CAD build for the part. Positions are in the model's coordinates, mm. Coordinates: 2 decimals unless noted, no trailing zeros. Order: outer loops, then holes, each group sorted by start corner. A loop starts at its lowest first (then second) coordinate and runs counter-clockwise, first axis right, second up. Notation, with made-up numbers: (29.5, -15) - (38.5, -15) arc R26 ccw to (38.5, -1) - close; hole circle Ø1 at (-38.75, -6). An arc over 180 degrees is marked (long way). Write each question's results on one line, items separated by ' | '. Start each with the question number.
Q1. Band-saw the part on C-C, the plane z = 1.2. Write the cut outline in (x, y), then the cut area to 3 significant figures.
Q2. Band-saw the part on A-A, the plane x = -88. Write the cut outline in (y, z).
Q3. Band-saw the part on B-B, the plane y = 0. Write the cut outline in (x, z).
Q4. Wall check: probe 1 along Y at (x, z) = (-40, 1.5); probe 2 along Y at (x, z) = (-70.5, 1.1); probe 3 along X at (y, z) = (-0.5, 0.35). Give the ranges that are in metal, low to high.
Q5. Band-saw the part on D-D, the plane x = -40. Write the cut outline in (y, z), then the cut area to 3 significant figures.
Q6. Pin check, flat tips, straight feed: P1, Ø10.5, axis at x = 40, y = 0, coming from the -Z side; P2, Ø7, axis at x = -40, y = 0, coming from the +Z side. Stop position of each tip, or through.
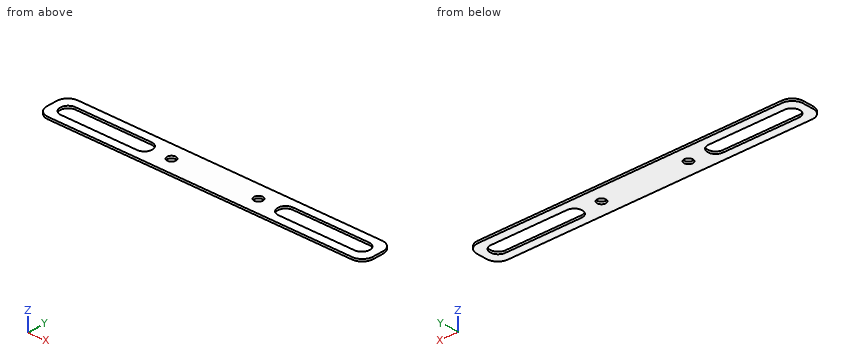
```python
from build123d import *

# Parameters (mm, degrees)
SKETCH1_W           = 300
SKETCH1_H           = 30
BOSS_EXTRUDE1_DEPTH = 2
CUT_EXTRUDE1_DEPTH  = 151.761400896
FILLET1_R           = 10
FILLET2_R           = 10
SKETCH4_R           = 4
CUT_EXTRUDE2_DEPTH  = 151.761400896


with BuildPart() as part:
    # Sketch1 → Boss-Extrude1 (new body)
    with BuildSketch(Plane.XY):
        Rectangle(SKETCH1_W, SKETCH1_H)
    extrude(amount=BOSS_EXTRUDE1_DEPTH)

    # Sketch2 → Cut-Extrude1 (cut, through all)
    with BuildSketch(Plane.XY.offset(2)):
        with BuildLine():
            Line((-135, 7.2), (-65, 7.2))
            ThreePointArc((-65, 7.2), (-57.8, 0), (-65, -7.2))
            Line((-65, -7.2), (-135, -7.2))
            ThreePointArc((-135, -7.2), (-142.2, 0), (-135, 7.2))
        make_face()
    cut_extrude1 = extrude(amount=-CUT_EXTRUDE1_DEPTH, mode=Mode.SUBTRACT)

    # Fillet1
    fillet1_edges = [part.edges().sort_by_distance(p)[0] for p in [
        (-150, 15, 1),
        (-150, -15, 1),
    ]]
    fillet(fillet1_edges, radius=FILLET1_R)

    # Mirror1: Cut-Extrude1 across plane
    add(cut_extrude1.mirror(Plane(origin=(0, 0, 0), x_dir=(0, 0, 1), z_dir=(1, 0, 0))), mode=Mode.SUBTRACT)

    # Fillet2
    fillet2_edges = [part.edges().sort_by_distance(p)[0] for p in [
        (150, 15, 1),
        (150, -15, 1),
    ]]
    fillet(fillet2_edges, radius=FILLET2_R)

    # Sketch4 → Cut-Extrude2 (cut, through all)
    with BuildSketch(Plane(origin=(0, 0, 0), x_dir=(-1, 0, 0), z_dir=(0, 0, -1))):
        with Locations((40, 0)):
            Circle(SKETCH4_R)
        with Locations((-40, 0)):
            Circle(SKETCH4_R)
    extrude(amount=-CUT_EXTRUDE2_DEPTH, mode=Mode.SUBTRACT)


solid = part.part
```
Results below:
1) outline: (-150, -5) arc R10 ccw to (-140, -15) - (140, -15) arc R10 ccw to (150, -5) - (150, 5) arc R10 ccw to (140, 15) - (-140, 15) arc R10 ccw to (-150, 5) - close; hole (-135, -7.2) - (-65, -7.2) arc R7.2 ccw to (-65, 7.2) - (-135, 7.2) arc R7.2 ccw to start; hole circle Ø8 at (-40, 0); hole circle Ø8 at (40, 0); hole (65, -7.2) - (135, -7.2) arc R7.2 ccw to (135, 7.2) - (65, 7.2) arc R7.2 ccw to start | area: 6,470 mm²
2) outline: (-15, 0) - (-7.2, 0) - (-7.2, 2) - (-15, 2) - close; (7.2, 0) - (15, 0) - (15, 2) - (7.2, 2) - close
3) outline: (-150, 0) - (-142.2, 0) - (-142.2, 2) - (-150, 2) - close; (-57.8, 0) - (-44, 0) - (-44, 2) - (-57.8, 2) - close; (-36, 0) - (36, 0) - (36, 2) - (-36, 2) - close; (44, 0) - (57.8, 0) - (57.8, 2) - (44, 2) - close; (142.2, 0) - (150, 0) - (150, 2) - (142.2, 2) - close
4) probe 1: y = -15 to -4, 4 to 15 | probe 2: y = -15 to -7.2, 7.2 to 15 | probe 3: x = -150 to -142.18, -57.82 to -43.97, -36.03 to 36.03, 43.97 to 57.82, 142.18 to 150
5) outline: (-15, 0) - (-4, 0) - (-4, 2) - (-15, 2) - close; (4, 0) - (15, 0) - (15, 2) - (4, 2) - close | area: 44.0 mm²
6) P1: stops at z = 0 | P2: passes through
